```python
from build123d import *

# Parameters (mm, degrees)
SKETCH1_R           = 7
BOSS_EXTRUDE1_DEPTH = 8


with BuildPart() as part:
    # Sketch1 → Boss-Extrude1 (new body)
    with BuildSketch(Plane.XY):
        with BuildLine():
            Line((10, 0), (90, 0))
            Line((90, 0), (210, 150))
            Line((210, 150), (210, 230))
            ThreePointArc((210, 230), (192.5, 247.5), (175, 230))
            Line((175, 230), (175, 200))
            ThreePointArc((175, 200), (150, 175), (125, 200))
            Line((125, 200), (125, 230))
            ThreePointArc((125, 230), (122.071067812, 237.071067812), (115, 240))
            Line((115, 240), (80, 240))
            Line((80, 240), (0, 160))
            Line((0, 160), (0, 10))
            ThreePointArc((0, 10), (2.928932188, 2.928932188), (10, 0))
        make_face()
        with Locations((40, 130)):
            Circle(SKETCH1_R, mode=Mode.SUBTRACT)
        with Locations((40, 30)):
            Circle(SKETCH1_R, mode=Mode.SUBTRACT)
    extrude(amount=BOSS_EXTRUDE1_DEPTH)


solid = part.part
```
The listing builds one solid part. Answer for the finished solid, in the listing's coordinates (mm). A direction names the side the tool comes from. Round coordinates to 2 decimals unless told otherwise and drop trailing zeros. Write each loop counter-clockwise with the first axis right and the second up, starting at its lowest first coordinate (ties: lowest second). Pieces come first, ordered by that corner, then holes. Notation, with made-up numbers: (28.5, -3) -> (69.5, -3) arc R28 cw to (69.5, 16) -> close; hole circle Ø6 at (86.5, 25.25). An arc over 180 degrees is marked (long way). Answer as a JSON object with one key per item and string values. Group by question number.
Q1. Each of these flat-tipped pins is pushed along its axis until it touches: pin 1 Ø2 at (y, z) = (45.5, 3) entering from +X; pin 2 Ø4 at (y, z) = (211.5, 3) entering from -X; pin 3 Ø4 at (x, z) = (158, 1) entering from -Y. Where does it stop, or does it pass through?
Q2. Straight lines are drawn through the part: line 1 along Y through (x, z) = (40, 5.75); line 2 along Y through (x, z) = (80, 5.5); line 3 along X through (y, z) = (127, 0.5). For each, find the intervals that lie inside material, in ascending order.
Q3. Section A-A (z = 2.75) is taken. Write down the section's boundary in (x, y), plus the area to 3 significant figures.
Q4. Section C-C (y = 194.5) is taken. Write down the section's boundary in (x, z), plus the area to 3 significant figures.
Q5. Determine the mould class of faces 4 (the face through (80, 125, 0)), 5 (the face through (149.2, 74, 3.9)), 6 (the face through (125, 215, 4)) for opening direction X: pulls with the +X half, pulls with the -X half, needs draft (parallel to the pull), parting line crosses it, or undercut.
Q6. Which of the six approach directions +Z, -Z, +X, -X, +Y, -Y give full straight-line access (tool end or side, diameter ignored) to faces 1 (the face through (175, 215, 4)), 2 (the face through (49, 0, 4)), 3 (the face through (98, 240, 4))?
Q7. Section B-B (x = 40) is taken. Write down the section's boundary in (y, z), plus the area to 3 significant figures.
Q8. Section D-D (x = 109) is taken. Write down the section's boundary in (y, z).
Check values:
{
 "1": {"pin 1": "x = 127.2", "pin 2": "x = 49.5", "pin 3": "y = 82.5"},
 "2": {"line 1": "0 to 23, 37 to 123, 137 to 200", "line 2": "0 to 240", "line 3": "0 to 33.68, 46.32 to 191.6"},
 "3": {"outline": "(0, 10) arc R10 ccw to (10, 0) -> (90, 0) -> (210, 150) -> (210, 230) arc R17.5 ccw to (175, 230) -> (175, 200) arc R25 cw to (125, 200) -> (125, 230) arc R10 ccw to (115, 240) -> (80, 240) -> (0, 160) -> close; hole circle Ø14 at (40, 30); hole circle Ø14 at (40, 130)", "area": "35,000 mm^2"},
 "4": {"outline": "(34.5, 0) -> (125.61, 0) -> (125.61, 8) -> (34.5, 8) -> close; (174.39, 0) -> (210, 0) -> (210, 8) -> (174.39, 8) -> close", "area": "1,010 mm^2"},
 "5": {"face 4": "needs draft", "face 5": "pulls with the +X half", "face 6": "undercut"},
 "6": {"face 1": "+Z, -Z, +Y", "face 2": "+Z, -Z, +X, -X, -Y", "face 3": "+Z, -Z, -X, +Y"},
 "7": {"outline": "(0, 0) -> (23, 0) -> (23, 8) -> (0, 8) -> close; (37, 0) -> (123, 0) -> (123, 8) -> (37, 8) -> close; (137, 0) -> (200, 0) -> (200, 8) -> (137, 8) -> close", "area": "1,380 mm^2"},
 "8": {"outline": "(23.75, 0) -> (240, 0) -> (240, 8) -> (23.75, 8) -> close"}
}
